The figure shows three views and two pictorial views of one solid part (mm, origin at its lowest corner). Answer the questions. A direction names the side the tool comes from. Give positions to 0.01 mm unless a question says otherwise; leave off trailing zeros. Loops run counter-clockwise (first coordinate to the right, second up) from the corner with the lowest first, then second, coordinate; pieces in that order, holes last. Notation, with made-up numbers: M 50.25,89.25 L 75.25,89.25 A7 ccw 75.25,100.25 Z; hole C -30.5,3 d4. An arc over 180 degrees is marked long. One line per item, written item: value. Start each with the question number.
Q1. A cutting plane is placed at C-C, the plane y = 2. Determine the outline of the cut face in (x, z).
Q2. For the marked faces 1, 2 and 3, determine the directions among +Z, -Z, +X, -X, +Y, -Y from which every point of the face is accessible in a straight line to the end or side of a thin tool.
Q3. Consider L1, parallel to Y at x = 23, z = 85; L2, parallel to X at y = 6.75, z = 11.5; L3, parallel to Z at x = 26.5, y = 2. Determine where each line is inside the solid, lowest interval first.
Q4. Flat-ended cylindrical pins translate along their axes: pin 1 (2 mm diameter, centred on y = 5, z = 95, fed in from +X); pin 2 (1 mm diameter, centred on y = 8.5, z = 76.5, fed in from +X); pin 3 (1 mm diameter, centred on y = 6.5, z = 33, fed in from -X); pin 4 (3 mm diameter, centred on x = 27.5, y = 5, fed in from +Z). Find the tip coordinate at first contact, or state that the pin passes through.
Q5. A cutting plane is placed at B-B, the plane x = 6. Determine the outline of the cut face in (y, z).
Q6. A cutting plane is placed at A-A, the plane z = 45. Determine the outline of the cut face in (x, y).
Q7. A cutting plane is placed at D-D, the plane z = 30.5. Determine the outline of the cut face in (x, y).
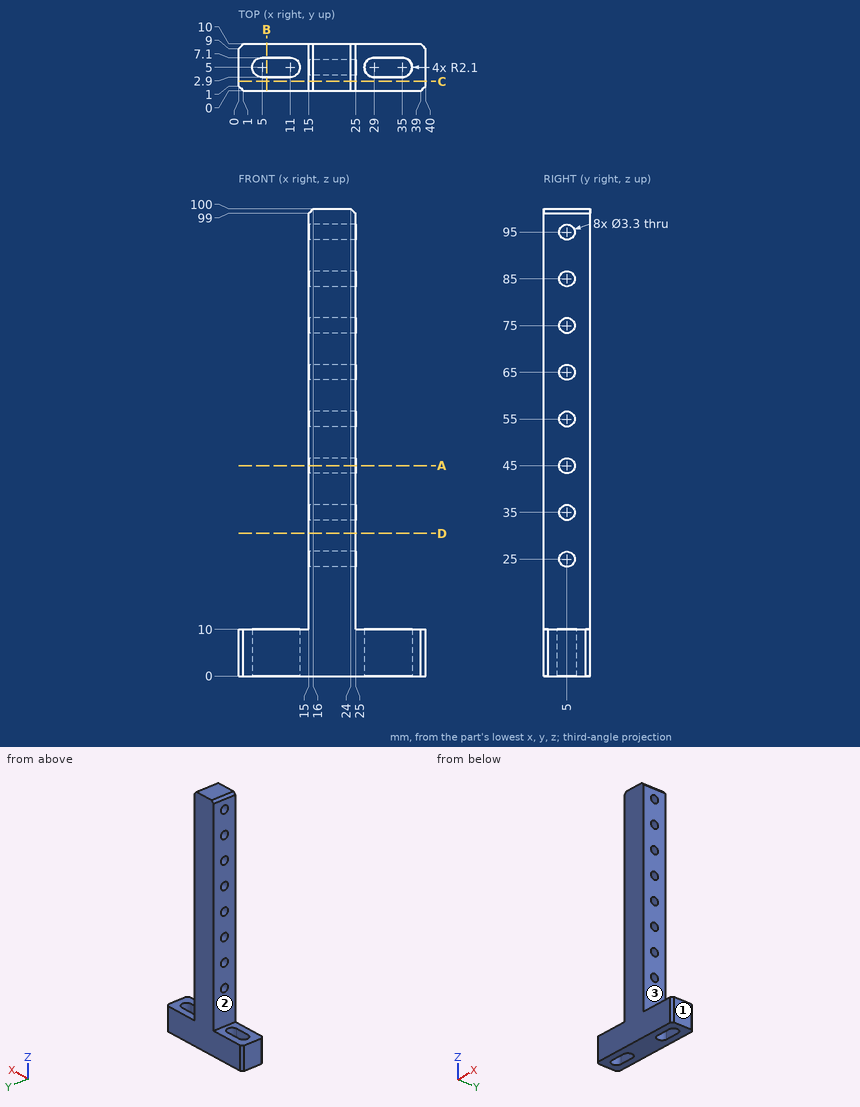
Answer block:
1. outline: M 0,0 L 40,0 L 40,10 L 25,10 L 25,99 L 24,100 L 16,100 L 15,99 L 15,10 L 0,10 Z
2. face 1: +Z, -Z, +X, +Y, -Y
2. face 2: +Z, -X, +Y, -Y
2. face 3: +Z, +X, +Y, -Y
3. L1: 0 to 3.35, 6.65 to 10
3. L2: 15 to 25
3. L3: 0 to 10
4. pin 1: through
4. pin 2: x = 25
4. pin 3: x = 15
4. pin 4: z = 10
5. outline: M 0,0 L 2.9,0 L 2.9,10 L 0,10 Z; M 7.1,0 L 10,0 L 10,10 L 7.1,10 Z
6. outline: M 15,0 L 25,0 L 25,3.35 L 15,3.35 Z; M 15,6.65 L 25,6.65 L 25,10 L 15,10 Z
7. outline: M 15,0 L 25,0 L 25,10 L 15,10 Z
